```python
from build123d import *

# Parameters (mm, degrees)
SKETCH1_R           = 45
SKETCH1_R_2         = 40
BOSS_EXTRUDE1_DEPTH = 50
SKETCH2_W           = 5
SKETCH2_H           = 40
CUT_EXTRUDE1_DEPTH  = 661.757616096
CIRPATTERN1_COUNT   = 8


with BuildPart() as part:
    # Sketch1 → Boss-Extrude1 (new body)
    with BuildSketch(Plane.XY):
        with Locations((-599.884196758, -90)):
            Circle(SKETCH1_R)
        with Locations((-599.884196758, -90)):
            Circle(SKETCH1_R_2, mode=Mode.SUBTRACT)
    extrude(amount=BOSS_EXTRUDE1_DEPTH)

    # Sketch2 → Cut-Extrude1 (cut, symmetric)
    with BuildSketch(Plane(origin=(0, 0, 0), x_dir=(1, 0, 0), z_dir=(0, 1, 0))):
        with Locations((-599.884196758, -25)):
            Rectangle(SKETCH2_W, SKETCH2_H)
    cut_extrude1 = extrude(amount=CUT_EXTRUDE1_DEPTH, both=True, mode=Mode.SUBTRACT)

    # CirPattern1: Cut-Extrude1 ×8 about axis
    cirpattern1_axis = Axis((-599.884196758, -90, 0), (0, 0, 1))
    for i in range(1, CIRPATTERN1_COUNT):
        add(cut_extrude1.rotate(cirpattern1_axis, i * 360 / CIRPATTERN1_COUNT), mode=Mode.SUBTRACT)


solid = part.part
```
Verification items for the finished model (mm, model axes). A direction names the side the tool comes from. Give positions to 0.01 mm unless a question says otherwise; leave off trailing zeros. Order: outer loops, then holes, each group sorted by start corner. A loop starts at its lowest first (then second) coordinate and runs counter-clockwise, first axis right, second up. Notation, with made-up numbers: (-26, 9) -> (33, 9) arc R23 cw to (33, 29) -> close; hole circle Ø7 at (77.5, 39.25). An arc over 180 degrees is marked (long way). Use a Markdown table: item, result.
1) Section check A-A, the plane y = -90. Record the boundary of the cut face in (x, z), then the cut area to 3 significant figures.
Results:
| item | result |
|---|---|
| outline | (-644.88, 0) -> (-639.88, 0) -> (-639.88, 5) -> (-644.88, 5) -> close; (-644.88, 45) -> (-639.88, 45) -> (-639.88, 50) -> (-644.88, 50) -> close; (-559.88, 0) -> (-554.88, 0) -> (-554.88, 5) -> (-559.88, 5) -> close; (-559.88, 45) -> (-554.88, 45) -> (-554.88, 50) -> (-559.88, 50) -> close |
| area | 100 mm² |
2) Material ranges on probe 1 along Y at (x, z) = (-589, 20); probe 2 along X at (y, z) = (-110, 23.5); probe 3 along Y at (x, z) = (-631, 34.5), recorded low to high.
Results:
| item | result |
|---|---|
| probe 1 | -133.66 to -128.49, -51.51 to -46.34 |
| probe 2 | -640.2 to -634.53, -565.24 to -559.57 |
| probe 3 | -117.58 to -115.14, -64.86 to -62.42 |
3) Tool access check on faces 1 (the flat face through (-600, -48, 5)), 2 (the flat face through (-630, -120, 45)), 3 (the flat face through (-642, -90, 5)). Record the directions out of +Z, -Z, +X, -X, +Y, -Y that give a thin tool (end or side, any length) a straight path to the whole face; none if there is none.
Results:
| item | result |
|---|---|
| face 1 | +Y, -Y |
| face 2 | none |
| face 3 | +X, -X |
4) Section check D-D, the plane y = -71. Record the boundary of the cut face in (x, z).
Results:
| item | result |
|---|---|
| outline | (-640.68, 0) -> (-635.08, 0) -> (-635.08, 50) -> (-640.68, 50) -> close; (-564.68, 0) -> (-559.09, 0) -> (-559.09, 50) -> (-564.68, 50) -> close |
5) Section check C-C, the plane x = -591. Record the boundary of the cut face in (y, z).
Results:
| item | result |
|---|---|
| outline | (-134.11, 0) -> (-129, 0) -> (-129, 50) -> (-134.11, 50) -> close; (-51, 0) -> (-45.89, 0) -> (-45.89, 50) -> (-51, 50) -> close |
6) Mould release check, pull along X, two halves, no side actions. Record for faces 4 (the flat face through (-631.68, -61.74, 25.28)), 5 (the cylindrical face through (-558.3, -107.2, 24.6)), 6 (the flat face through (-642, -92.5, 25)): pulls with the +X half, pulls with the -X half, needs draft (parallel to the pull), parting line crosses it, or undercut.
Results:
| item | result |
|---|---|
| face 4 | undercut |
| face 5 | parting line crosses it |
| face 6 | needs draft |
7) Section check B-B, the plane z = 20. Give the number of separate pieces and of enclosed holes in the cut face, then the cut area to 3 significant figures.
Results:
| item | result |
|---|---|
| separate pieces | 8 |
| enclosed holes | 0 |
| area | 1,140 mm² |
8) Depth check by flat-ended pin: pin 1 Ø1.5 at (y, z) = (-90.5, 14) entering from +X; pin 2 Ø5 at (x, z) = (-592, 27.5) entering from -Y; pin 3 Ø4 at (x, z) = (-589, 29) entering from +Y; pin 4 Ø4 at (x, z) = (-634, 39) entering from +Y. Enter the tip coordinate at first touch or a pass-through.
Results:
| item | result |
|---|---|
| pin 1 | through |
| pin 2 | y = -134.68 |
| pin 3 | y = -45.89 |
| pin 4 | y = -60 |
